Can you work these out from the model? Positions are in its coordinate system, mm. Round coordinates to 2 decimals unless told otherwise and drop trailing zeros. Loops run counter-clockwise (first coordinate to the right, second up) from the corner with the lowest first, then second, coordinate; pieces in that order, holes last.
from build123d import *

# Parameters (mm, degrees)
SKETCH_1_W                = 850
SKETCH_1_H                = 950
EXTRUDE_1_DEPTH           = 15
FILLET_1_R                = 5
HOLE_WIZARD_M5_1_D        = 4.2
PATTERN_LINEAR_1_COUNT    = 5
PATTERN_LINEAR_1_PITCH    = 100
HOLE_WIZARD_M6_1_D        = 5
CUT_EXTRUDE_1_REACH       = 639.554
SKETCH_6_R                = 40
HOLE_WIZARD_M5_2_D        = 4.2
HOLE_WIZARD_1_D           = 6.6
HOLE_WIZARD_1_CBORE_D     = 11
HOLE_WIZARD_1_CBORE_DEPTH = 6.8
HOLE_WIZARD_M6_2_D        = 5


with BuildPart() as part:
    # 草图1 → 凸台-拉伸1 (new body)
    with BuildSketch(Plane.XY):
        Rectangle(SKETCH_1_W, SKETCH_1_H)
    extrude(amount=EXTRUDE_1_DEPTH)

    # 圆角1
    fillet_1_edges = [part.edges().sort_by_distance(p)[0] for p in [
        (-425, 475, 7.5),
        (425, 475, 7.5),
        (425, -475, 7.5),
        (-425, -475, 7.5),
    ]]
    fillet(fillet_1_edges, radius=FILLET_1_R)

    # M5 螺纹孔1 (through all)
    with Locations(Plane.XY.offset(15)):
        with Locations((265, -140.199999647), (265, -208.199999647)):
            hole_wizard_m5_1 = Hole(HOLE_WIZARD_M5_1_D / 2)

    # 阵列(线性)1: M5 螺纹孔1 ×5
    with Locations(*[(-i * PATTERN_LINEAR_1_PITCH, 0, 0) for i in range(1, PATTERN_LINEAR_1_COUNT)]):
        add(hole_wizard_m5_1, mode=Mode.SUBTRACT)

    # M6 螺纹孔1 (through all)
    with Locations(Plane.XY.offset(15)):
        with Locations((-185, -3.399999647), (-65, -3.399999647), (55, -3.399999647), (175, -3.399999647), (295, -3.399999647)):
            Hole(HOLE_WIZARD_M6_1_D / 2)

    # 草图6 → 切除-拉伸1 (cut, up to next)
    with BuildSketch(Plane.XY.offset(15), mode=Mode.PRIVATE) as cut_extrude_1_sk1:
        with Locations((-275, -355)):
            Circle(SKETCH_6_R)
    cut_extrude_1_tool1 = extrude(cut_extrude_1_sk1.sketch, amount=-CUT_EXTRUDE_1_REACH, mode=Mode.PRIVATE) & part.part
    # 草图6 → 切除-拉伸1 (cut, up to next)
    with BuildSketch(Plane.XY.offset(15), mode=Mode.PRIVATE) as cut_extrude_1_sk2:
        with Locations((275, -355)):
            Circle(SKETCH_6_R)
    cut_extrude_1_tool2 = extrude(cut_extrude_1_sk2.sketch, amount=-CUT_EXTRUDE_1_REACH, mode=Mode.PRIVATE) & part.part
    add(cut_extrude_1_tool1.solids().sort_by_distance((-275, -355, 15))[0], mode=Mode.SUBTRACT)
    add(cut_extrude_1_tool2.solids().sort_by_distance((275, -355, 15))[0], mode=Mode.SUBTRACT)

    # M5 螺纹孔2 (through all)
    with Locations(Plane.XY.offset(15)):
        with Locations((-155, -248), (-155, -276.5), (-155, -305)):
            Hole(HOLE_WIZARD_M5_2_D / 2)

    # 打孔尺寸(%根据)内六角圆柱头螺钉的类型1 (through all)
    with Locations(Plane.XY.offset(15)):
        with Locations((-405, -455), (0, -455), (405, -455), (0, 0), (-405, 0), (-405, 455), (0, 455), (405, 455), (405, 0)):
            CounterBoreHole(HOLE_WIZARD_1_D / 2, HOLE_WIZARD_1_CBORE_D / 2, HOLE_WIZARD_1_CBORE_DEPTH)

    # M6 螺纹孔2 (through all)
    with Locations(Plane.XY.offset(15)):
        with Locations((-405, 200), (-405, -200), (-200, -455), (200, -455), (405, -200), (405, 200), (200, 455), (-200, 455)):
            Hole(HOLE_WIZARD_M6_2_D / 2)


solid = part.part
(1) Will this pin go through, and if not, where does the flat tip stop? P1, Ø10, axis at x = -405, y = -455, coming from the -Z side.
Worked answers:
P1: stops at z = 0
(2) If we mould it in two halves opening along X, with no side actions, what happens to faces 1 (the cylindrical face through (245.518, -327.966, 7.605)), 2 (the flat face through (-6, 7, 15))? For each: released by +X, released by -X, zero draft, split by the parting line, or undercut.
Worked answers:
face 1: undercut
face 2: zero draft
(3) If I drill on line 1 (Y direction, x = -155, z = 8.75); line 2 (X direction, y = -200, z = 7); line 3 (X direction, y = -455, z = 10.5), over which ranges is the centre line in solid material (lowest first)?
Worked answers:
line 1: y = -475 to -307.1, -302.9 to -278.6, -274.4 to -250.1, -245.9 to 475
line 2: x = -425 to -407.5, -402.5 to 402.5, 407.5 to 425
line 3: x = -425 to -410.5, -399.5 to -202.5, -197.5 to -5.5, 5.5 to 197.5, 202.5 to 399.5, 410.5 to 425
(4) If we section it at A-A, the plane x = -275: List the corners of the cut face in (y, z) for me.
Worked answers:
outline: (-475, 0) - (-395, 0) - (-395, 15) - (-475, 15) - close; (-315, 0) - (475, 0) - (475, 15) - (-315, 15) - close
